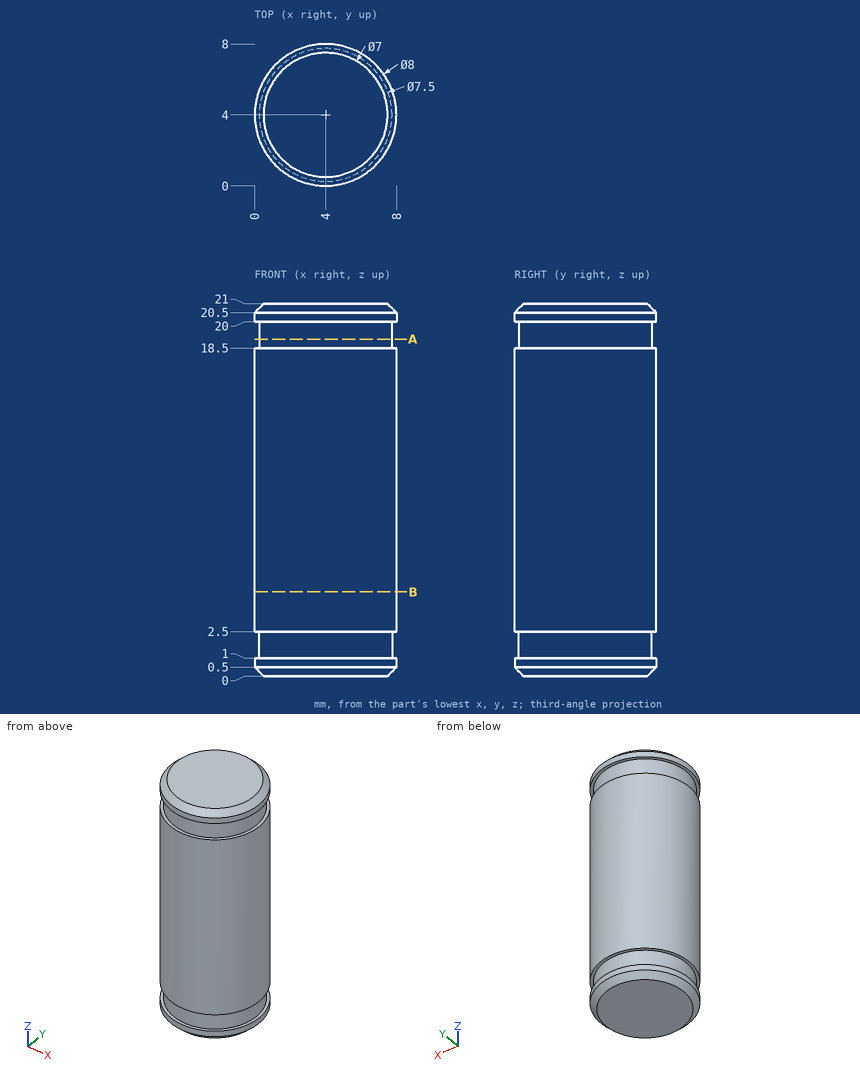
Check sheet for the drawn part. Datum: minimum x, y, z corner. Units: mm. Give positions to 0.01 mm unless a question says otherwise; leave off trailing zeros. Order: outer loops, then holes, each group sorted by start corner. A loop starts at its lowest first (then second) coordinate and runs counter-clockwise, first axis right, second up. Notation, with made-up numbers: (12, 48) - (61, 48) arc R24 ccw to (61, 84) - close; hole circle Ø4 at (-7.75, 14.25). An arc over 180 degrees is marked (long way). Answer as a JSON object with one key per item and string values.
(1) Cross-section at A-A (z = 19). Record the cut outline in (x, y), then the cut area to 3 significant figures.
Report:
{"outline": "circle Ø7.5 at (4, 4)", "area": "44.2 mm^2"}
(2) Material ranges on line 1 (Y direction, x = 7.25, z = 19.5); line 2 (X direction, y = 6.5, z = 18); line 3 (X direction, y = 6, z = 12.25), recorded low to high.
Report:
{"line 1": "2.13 to 5.87", "line 2": "0.88 to 7.12", "line 3": "0.54 to 7.46"}
(3) Cross-section at B-B (z = 4.75). Record the cut outline in (x, y), then the cut area to 3 significant figures.
Report:
{"outline": "circle Ø8 at (4, 4)", "area": "50.3 mm^2"}
(4) Depth check by flat-ended pin: pin 1 Ø1.5 at (y, z) = (3, 10) entering from -X. Enter the tip coordinate at first touch or a pass-through.
Report:
{"pin 1": "x = 0.01"}
